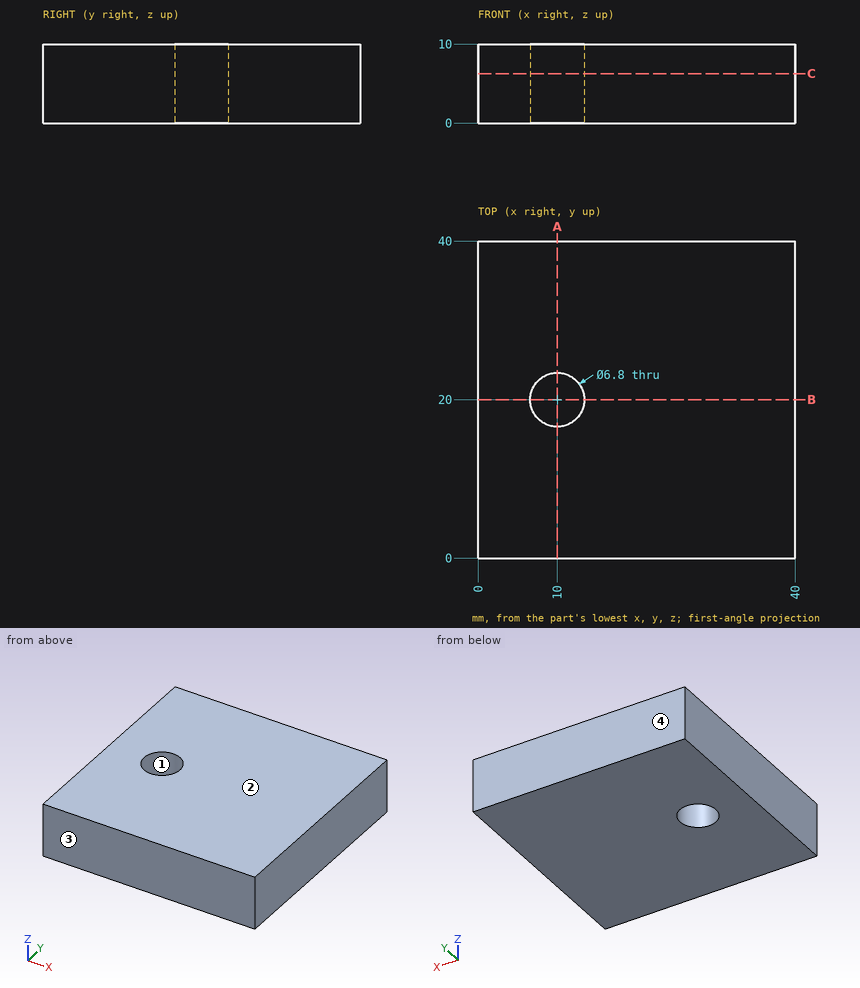
Answer from the drawing. Dimensions are ordinates in mm from the lowest x, y and z of the part. Round coordinates to 2 decimals unless told otherwise and drop trailing zeros. Order: outer loops, then holes, each group sorted by start corner. A loop starts at its lowest first (then second) coordinate and runs counter-clockwise, first axis right, second up. Notation, with made-up numbers: (-21, -29.75) - (12, -29.75) arc R21 ccw to (12, -23.75) - close; hole circle Ø2 at (-2.75, -34.75). An arc over 180 degrees is marked (long way). Put each result on its own line as item: value. Start each with the question number.
(1) Determine the mould class of the marked faces 1, 2, 3 and 4 for opening direction Y: released by +Y, released by -Y, zero draft, split by the parting line, or undercut.
(2) Find section C-C (z = 6.25). Give the vertices of the cut face in (x, y).
(3) Find section A-A (x = 10). Give the vertices of the cut face in (y, z).
(4) Find section B-B (y = 20). Give the vertices of the cut face in (x, z), plus the area to 3 significant figures.
(5) Straight lines are drawn through the part: probe 1 along Y at (x, z) = (10, 6); probe 2 along X at (y, z) = (19, 9); probe 3 along Y at (x, z) = (11, 5.25). For each, find the intervals that lie inside material, in ascending order. Write a range as from..to.
Reply:
1. face 1: undercut
1. face 2: zero draft
1. face 3: released by -Y
1. face 4: released by +Y
2. outline: (0, 0) - (40, 0) - (40, 40) - (0, 40) - close; hole circle Ø6.8 at (10, 20)
3. outline: (0, 0) - (16.6, 0) - (16.6, 10) - (0, 10) - close; (23.4, 0) - (40, 0) - (40, 10) - (23.4, 10) - close
4. outline: (0, 0) - (6.6, 0) - (6.6, 10) - (0, 10) - close; (13.4, 0) - (40, 0) - (40, 10) - (13.4, 10) - close
4. area: 332 mm^2
5. probe 1: 0..16.6, 23.4..40
5. probe 2: 0..6.75, 13.25..40
5. probe 3: 0..16.75, 23.25..40
